```python
from build123d import *

# Parameters (mm, degrees)
SKETCH_1_R          = 32
EXTRUDE_1_DEPTH     = 25
CUT_EXTRUDE_1_DEPTH = 52.701063819
SKETCH_3_R          = 21.5
CUT_EXTRUDE_2_DEPTH = 10
CHAMFER_1_SIZE      = 2


with BuildPart() as part:
    # 草图1 → 凸台-拉伸1 (new body)
    with BuildSketch(Plane.XY):
        Circle(SKETCH_1_R)
    extrude(amount=EXTRUDE_1_DEPTH)

    # 草图2 → 切除-拉伸1 (cut, through all)
    with BuildSketch(Plane.XY.offset(25)):
        Polygon((17.320508076, 0), (8.660254038, 15), (-8.660254038, 15), (-17.320508076, 0), (-8.660254038, -15), (8.660254038, -15), align=None)
    extrude(amount=-CUT_EXTRUDE_1_DEPTH, mode=Mode.SUBTRACT)

    # 草图3 → 切除-拉伸2 (cut)
    with BuildSketch(Plane(origin=(0, 0, 0), x_dir=(-1, 0, 0), z_dir=(0, 0, -1))):
        Circle(SKETCH_3_R)
    extrude(amount=-CUT_EXTRUDE_2_DEPTH, mode=Mode.SUBTRACT)

    # 倒角1
    chamfer_1_edges = [part.edges().sort_by_distance(p)[0] for p in [
        (-32, 0, 0),
    ]]
    chamfer(chamfer_1_edges, length=CHAMFER_1_SIZE)


solid = part.part
```
Read the model definition and answer for the solid it produces. Units are mm, in the model's axes. A direction names the side the tool comes from. Coordinates: 2 decimals unless noted, no trailing zeros. Write each loop counter-clockwise with the first axis right and the second up, starting at its lowest first coordinate (ties: lowest second). Pieces come first, ordered by that corner, then holes. Notation, with made-up numbers: (82.5, -15.75) - (89.5, -15.75) arc R26 cw to (89.5, 18.25) - close; hole circle Ø6 at (52.5, 77). An arc over 180 degrees is marked (long way). Answer as a JSON object with one key per item and string values. Group by question number.
1. A cutting plane is placed at A-A (x = 0). Determine the outline of the cut face in (y, z), plus the area to 3 significant figures.
2. Each of these flat-tipped pins is pushed along its axis until it touches: P1, Ø6, axis at y = -16, z = 21, coming from the -X side; P2, Ø12, axis at x = 2, z = 19.5, coming from the -Y side; P3, Ø5, axis at x = 16, z = 13, coming from the -Y side. Where does it stop, or does it pass through?
3. A cutting plane is placed at B-B (z = 14). Determine the outline of the cut face in (x, y).
4. Consider L1, parallel to Y at x = 0, z = 3.5; L2, parallel to Y at x = 2, z = 3; L3, parallel to Z at x = 0, y = 17.5. Determine where each line is inside the solid, lowest interval first. Write a range as [from, to].
5. The mould has two halves that part along Y. Classify faces 4 (the cylindrical face through (2.799, 21.317, 4.93)), 5 (the flat face through (14, -7, 25)), 6 (the cylindrical face through (-6.94, -31.24, 13.34)): +Y half, -Y half, draft (parallel to the pull), parting line (faces both ways), or undercut.
6. A cutting plane is placed at C-C (z = 6). Determine the outline of the cut face in (x, y).
7. Which of the six approach directions +Z, -Z, +X, -X, +Y, -Y give full straight-line access (tool end or side, diameter ignored) to faces 1 (the flat face through (20, -13, 0)), 2 (the flat face through (-13.05, -7.4, 17.6)), 3 (the flat face through (13, -8, 10))?
Worked out:
{
 "1": {"outline": "(-32, 2) - (-30, 0) - (-21.5, 0) - (-21.5, 10) - (-15, 10) - (-15, 25) - (-32, 25) - close; (15, 10) - (21.5, 10) - (21.5, 0) - (30, 0) - (32, 2) - (32, 25) - (15, 25) - close", "area": "716 mm²"},
 "2": {"P1": "stops at x = -29.24", "P2": "stops at y = -32", "P3": "stops at y = -29.01"},
 "3": {"outline": "circle Ø64 at (0, 0); hole (-17.32, 0) - (-8.66, -15) - (8.66, -15) - (17.32, 0) - (8.66, 15) - (-8.66, 15) - close"},
 "4": {"L1": "y = [-32, -21.5], [21.5, 32]", "L2": "y = [-31.94, -21.41], [21.41, 31.94]", "L3": "z = [10, 25]"},
 "5": {"face 4": "undercut", "face 5": "draft", "face 6": "parting line"},
 "6": {"outline": "circle Ø64 at (0, 0); hole circle Ø43 at (0, 0)"},
 "7": {"face 1": "-Z, +X, -X, +Y, -Y", "face 2": "+Z, -Z", "face 3": "-Z"}
}
